Work out the finished part from the listing and answer in its coordinate system (mm). A direction names the side the tool comes from. Give positions to 0.01 mm unless a question says otherwise; leave off trailing zeros. Write each loop counter-clockwise with the first axis right and the second up, starting at its lowest first coordinate (ties: lowest second). Pieces come first, ordered by that corner, then holes. Notation, with made-up numbers: (32, 74.25) -> (82, 74.25) arc R23 cw to (82, 96.25) -> close; hole circle Ø6 at (-5, -40). An arc over 180 degrees is marked (long way). Use a Markdown table: item, result. Add a question column.
Q1. Each of these flat-tipped pins is pushed along its axis until it touches: pin 1 Ø5 at (x, z) = (24.5, 6) entering from +Y; pin 2 Ø2.5 at (x, z) = (0, -0.5) entering from +Y; pin 3 Ø1.8 at (x, z) = (-0.5, 9.5) entering from -Y; pin 4 Ø12 at (x, y) = (0, 0) entering from -Z. Where does it stop, or does it pass through?
Q2. Section B-B, the plane z = 0 is taken. Give the vertices of the cut face in (x, y), plus the area to 3 significant figures.
Q3. Section C-C, the plane y = 1 is taken. State how many separate pieces and enclosed holes the cut face has, plus the area to 3 significant figures.
Q4. For faces 5 (the face through (2.6, 12.8, 0.4)), 6 (the face through (-2.44, 27.1, -0.54)), 7 (the face through (-27.098, 0.751, 2.385)), determine the directions among +Z, -Z, +X, -X, +Y, -Y from which every point of the face is accessible in a straight line to the end or side of a thin tool.
Q5. Section A-A, the plane z = -18 is taken. Give the vertices of the cut face in (x, y).
Q6. Consider line 1 (X direction, y = 0, z = -14.5); line 2 (Z direction, x = 0, y = 18); line 3 (Z direction, x = 0, y = 25.25). Determine where each line is inside the solid, lowest interval first.
Q7. For a pull along Y with two mould halves and no side action, classify faces 1 (the face through (-24.3, 23.78, 0.03)), 2 (the face through (-3, 11, 0)), 3 (the face through (8, -8, 25)), 4 (the face through (-8.67, -39.05, -14.86)) as pulls with the +Y half, pulls with the -Y half, needs draft (parallel to the pull), parting line crosses it, or undercut.
from build123d import *
from build123d.topology import SkipClean

# Parameters (mm, degrees)
SKETCH_1_R               = 40
SKETCH_1_R_2             = 10
EXTRUDE_1_DEPTH          = 25
SKETCH_6_W               = 6
SKETCH_6_H               = 9.759677648
CUT_EXTRUDE_1_DEPTH      = 76.498344353
SKETCH_8_W               = 2.1
SKETCH_8_H               = 40
CUT_EXTRUDE_START        = 40
SKETCH_9_R               = 2.5
CUT_EXTRUDE_2_DEPTH      = 20
PATTERN_CIRCULAR_1_COUNT = 2
PATTERN_CIRCULAR_1_ANGLE = 90


with BuildPart() as part:
    # 草图1 → 凸台-拉伸1 (new, symmetric)
    with BuildSketch(Plane.XY):
        Circle(SKETCH_1_R)
        Circle(SKETCH_1_R_2, mode=Mode.SUBTRACT)
    extrude(amount=EXTRUDE_1_DEPTH, both=True)

    # 草图5 → 切除-旋转1 (revolve, cut)
    with BuildSketch(Plane(origin=(0, 0, 0), x_dir=(1, 0, 0), z_dir=(0, 1, 0)), mode=Mode.PRIVATE) as cut_revolve_1_sk:
        Polygon((-40, -5), (-40, 5), (-34, 2.5), (-34, -2.5), align=None)
    revolve(cut_revolve_1_sk.sketch.rotate(Axis((0, 0, 0), (0, 0, -1)), 180), axis=Axis((0, 0, 0), (0, 0, -1)), mode=Mode.SUBTRACT)

    # 草图6 → 切除-拉伸1 (cut, through all)
    with BuildSketch(Plane.XY.offset(25)):
        with Locations((0, 7.920161176)):
            Rectangle(SKETCH_6_W, SKETCH_6_H)
    extrude(amount=-CUT_EXTRUDE_1_DEPTH, mode=Mode.SUBTRACT)

    # 草图8 → M5 螺纹孔1 (revolve, cut)
    with BuildSketch(Plane(origin=(0, 0, 0), x_dir=(0, 0, -1), z_dir=(1, 0, 0))):
        with Locations((1.05, 20)):
            Rectangle(SKETCH_8_W, SKETCH_8_H)
    hole_wizard_m5_1 = revolve(axis=Axis((0, -6.35, 0), (0, 1, 0)), mode=Mode.SUBTRACT)

    # 草图9 → 切除-拉伸2 (cut)
    with SkipClean():  # the faces are left unmerged after this step: merging them gives an invalid solid
        with BuildSketch(Plane(origin=(0, 0, 0), x_dir=(1, 0, 0), z_dir=(0, 1, 0)).offset(CUT_EXTRUDE_START)):
            with Locations(Location((0, 0, 0), (0, 0, 270))):
                Circle(SKETCH_9_R)
        cut_extrude_2 = extrude(amount=-CUT_EXTRUDE_2_DEPTH, mode=Mode.SUBTRACT)

    # 阵列(圆周)1: M5 螺纹孔1, 切除-拉伸2 ×2 about axis
    pattern_circular_1_axis = Axis((0, 0, 25), (0, 0, 1))
    add([hole_wizard_m5_1.rotate(pattern_circular_1_axis, i * PATTERN_CIRCULAR_1_ANGLE / (PATTERN_CIRCULAR_1_COUNT - 1)) for i in range(1, PATTERN_CIRCULAR_1_COUNT)], mode=Mode.SUBTRACT)
    add([cut_extrude_2.rotate(pattern_circular_1_axis, i * PATTERN_CIRCULAR_1_ANGLE / (PATTERN_CIRCULAR_1_COUNT - 1)) for i in range(1, PATTERN_CIRCULAR_1_COUNT)], mode=Mode.SUBTRACT)


solid = part.part
Result set:
| question | item | result |
|---|---|---|
| 1 | pin 1 | stops at y = 33.41 |
| 1 | pin 2 | stops at y = -9.92 |
| 1 | pin 3 | stops at y = -40 |
| 1 | pin 4 | passes through |
| 2 | outline | (-33.91, -2.5) arc R34 ccw (long way) to (2.5, 33.91) -> (2.5, 20) -> (2.1, 20) -> (2.1, 12.8) -> (3, 12.8) -> (3, 9.54) arc R10 cw (long way) to (-9.78, -2.1) -> (-20, -2.1) -> (-20, -2.5) -> close; (-33.91, 2.5) -> (-20, 2.5) -> (-20, 2.1) -> (-9.78, 2.1) arc R10 cw to (-3, 9.54) -> (-3, 12.8) -> (-2.1, 12.8) -> (-2.1, 20) -> (-2.5, 20) -> (-2.5, 33.91) arc R34 ccw to start |
| 2 | area | 3,090 mm2 |
| 3 | separate pieces | 3 |
| 3 | enclosed holes | 0 |
| 3 | area | 2,810 mm2 |
| 4 | face 5 | +Z, -Z |
| 4 | face 6 | +Y |
| 4 | face 7 | -X |
| 5 | outline | circle Ø80 at (0, 0); hole (-3, 9.54) arc R10 ccw (long way) to (3, 9.54) -> (3, 12.8) -> (-3, 12.8) -> close |
| 6 | line 1 | x = -40 to -10, 10 to 40 |
| 6 | line 2 | z = -25 to -2.1, 2.1 to 25 |
| 6 | line 3 | z = -25 to -2.5, 2.5 to 25 |
| 7 | face 1 | pulls with the +Y half |
| 7 | face 2 | undercut |
| 7 | face 3 | needs draft |
| 7 | face 4 | parting line crosses it |
